Build history of the part. All positions in model axes, mm. A direction names the side the tool comes from. Coordinates: 2 decimals unless noted, no trailing zeros. Write each loop counter-clockwise with the first axis right and the second up, starting at its lowest first coordinate (ties: lowest second). Pieces come first, ordered by that corner, then holes. Notation, with made-up numbers: M -34,86 L -19,86 A19 ccw -19,118 Z; hole C 9,-19 d2. An arc over 180 degrees is marked long. Use CSV: the item, a comma, the result in double quotes. Start each with the question number.
```python
from build123d import *

# Parameters (mm, degrees)
BOSS_EXTRUDE1_DEPTH = 10
SKETCH2_R           = 10
CUT_EXTRUDE1_DEPTH  = 222.133443875
SKETCH4_R           = 32.878916004
BOSS_EXTRUDE2_DEPTH = 10
SKETCH5_R           = 10
CUT_EXTRUDE3_DEPTH  = 227.48659951


with BuildPart() as part:
    # Sketch1 → Boss-Extrude1 (new body)
    with BuildSketch(Plane.XY):
        with BuildLine():
            Line((-200, 20), (200, 20))
            ThreePointArc((200, 20), (220, 0), (200, -20))
            Line((200, -20), (-200, -20))
            ThreePointArc((-200, -20), (-220, 0), (-200, 20))
        make_face()
    extrude(amount=BOSS_EXTRUDE1_DEPTH)

    # Sketch2 → Cut-Extrude1 (cut, through all)
    with BuildSketch(Plane.XY.offset(10)):
        with Locations((-200, 0)):
            Circle(SKETCH2_R)
        with Locations((200, 0)):
            Circle(SKETCH2_R)
    extrude(amount=-CUT_EXTRUDE1_DEPTH, mode=Mode.SUBTRACT)

    # Sketch4 → Boss-Extrude2 (add)
    with BuildSketch(Plane.XY.offset(10)):
        with Locations((0, 20)):
            Circle(SKETCH4_R)
    extrude(amount=-BOSS_EXTRUDE2_DEPTH)

    # Sketch5 → Cut-Extrude3 (cut, through all)
    with BuildSketch(Plane.XY.offset(10)):
        with Locations((0, 20)):
            Circle(SKETCH5_R)
    extrude(amount=-CUT_EXTRUDE3_DEPTH, mode=Mode.SUBTRACT)


solid = part.part
```
1. Flat gauge pins, fed straight in: pin 1 (5 mm diameter, centred on y = 36.5, z = 7, fed in from +X); pin 2 (18 mm diameter, centred on x = 0, y = 20, fed in from -Z); pin 3 (6 mm diameter, centred on x = -62.5, z = 4.5, fed in from +Y); pin 4 (1 mm diameter, centred on y = 29, z = 7, fed in from +X). Where does each tip first touch, or does it go through?
2. 3-axis set-ups, long thin cutter, end or side, ignore diameter. For faces 1 (the flat face through (-118, 20, 5)), 2 (the flat face through (-3, 1, 0)), 3 (the flat face through (115, 20, 5)): which of +Z, -Z, +X, -X, +Y, -Y reach the whole face in a straight line?
3. Pull direction Y, two halves, no side cores. Call faces 4 (the flat face through (3, -20, 5)), 5 (the cylindrical face through (220, 0, 5)), 6 (the cylindrical face through (209.237, -3.83, 5.07)): pulls with the +Y half, pulls with the -Y half, needs draft (parallel to the pull), parting line crosses it, or undercut.
4. Drill centre lines: line 1 along X through (y, z) = (-0.5, 4.75); line 2 along Y through (x, z) = (0, 4); line 3 along X through (y, z) = (4, 9.25). Where is each one in solid material? Low to high. Write a range as from..to.
5. Slice it at B-B (y = 0). List the corners of the cut face in (x, z).
6. Slice it at D-D (x = -172). List the corners of the cut face in (y, z).
7. Slice it at C-C (z = 4.75). List the corners of the cut face in (x, y).
8. Slice it at A-A (x = 0). List the corners of the cut face in (y, z), and give its area (3 significant figures).
Established:
1,pin 1,"stops at x = 29.75"
1,pin 2,"passes through"
1,pin 3,"stops at y = 20"
1,pin 4,"stops at x = 31.76"
2,face 1,"+Z, -Z, -X, +Y"
2,face 2,"-Z, +X, -X, +Y, -Y"
2,face 3,"+Z, -Z, +X, +Y"
3,face 4,"pulls with the -Y half"
3,face 5,"parting line crosses it"
3,face 6,"undercut"
4,line 1,"x = -219.99..-209.99, -190.01..190.01, 209.99..219.99"
4,line 2,"y = -20..10, 30..52.88"
4,line 3,"x = -219.6..-209.17, -190.83..190.83, 209.17..219.6"
5,outline,"M -220,0 L -210,0 L -210,10 L -220,10 Z; M -190,0 L 190,0 L 190,10 L -190,10 Z; M 210,0 L 220,0 L 220,10 L 210,10 Z"
6,outline,"M -20,0 L 20,0 L 20,10 L -20,10 Z"
7,outline,"M -200,-20 L 200,-20 A20 ccw 200,20 L 32.88,20 A32.88 ccw -32.88,20 L -200,20 A20 ccw Z; hole C -200,0 d20; hole C 0,20 d20; hole C 200,0 d20"
8,outline,"M -20,0 L 10,0 L 10,10 L -20,10 Z; M 30,0 L 52.88,0 L 52.88,10 L 30,10 Z"
8,area,"529 mm2"
